```python
from build123d import *

# Parameters (mm, degrees)
EXTRUDE_1_DEPTH     = 680
CUT_EXTRUDE_1_DEPTH = 683.878423476


with BuildPart() as part:
    # 草图1 → 凸台-拉伸1 (new body)
    with BuildSketch(Plane(origin=(0, 0, 0), x_dir=(1, 0, 0), z_dir=(0, 1, 0))):
        with BuildLine():
            Line((-19, -12.278106509), (19, -12.278106509))
            ThreePointArc((19, -12.278106509), (23.242640687, -10.520747196), (25, -6.278106509))
            Line((25, -6.278106509), (25, 31.721893491))
            ThreePointArc((25, 31.721893491), (23.242640687, 35.964534178), (19, 37.721893491))
            Line((19, 37.721893491), (-19, 37.721893491))
            ThreePointArc((-19, 37.721893491), (-23.242640687, 35.964534178), (-25, 31.721893491))
            Line((-25, 31.721893491), (-25, -6.278106509))
            ThreePointArc((-25, -6.278106509), (-23.242640687, -10.520747196), (-19, -12.278106509))
        make_face()
        with BuildLine():
            Line((-19, -7.278106509), (19, -7.278106509))
            ThreePointArc((19, -7.278106509), (19.707106781, -6.98521329), (20, -6.278106509))
            Line((20, -6.278106509), (20, 31.721893491))
            ThreePointArc((20, 31.721893491), (19.707106781, 32.429000272), (19, 32.721893491))
            Line((19, 32.721893491), (-19, 32.721893491))
            ThreePointArc((-19, 32.721893491), (-19.707106781, 32.429000272), (-20, 31.721893491))
            Line((-20, 31.721893491), (-20, -6.278106509))
            ThreePointArc((-20, -6.278106509), (-19.707106781, -6.98521329), (-19, -7.278106509))
        make_face(mode=Mode.SUBTRACT)
    extrude(amount=EXTRUDE_1_DEPTH)

    # 草图2 → 切除-拉伸1 (cut, through all)
    with BuildSketch(Plane(origin=(25, 0, 0), x_dir=(0, 0, -1), z_dir=(1, 0, 0))):
        Polygon((-12.278106509, 680), (37.721893491, 680), (37.721893491, 630), align=None)
        Polygon((-12.278106509, 0), (37.721893491, 50), (37.721893491, 0), align=None)
    extrude(amount=-CUT_EXTRUDE_1_DEPTH, mode=Mode.SUBTRACT)


solid = part.part
```
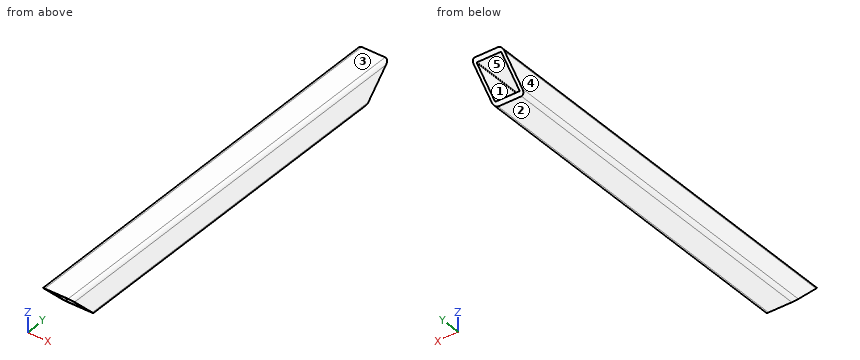
Here's how the part is built. I have some questions about the finished solid (model axes, mm). Face numbers are marked on the shaded views. A direction names the side the tool comes from. Round coordinates to 2 decimals unless told otherwise and drop trailing zeros. Order: outer loops, then holes, each group sorted by start corner. A loop starts at its lowest first (then second) coordinate and runs counter-clockwise, first axis right, second up. Notation, with made-up numbers: M 31,31.25 L 62,31.25 A23 cw 62,42.25 Z; hole C -26,23 d5. An arc over 180 degrees is marked long. Use CSV: the item, a comma, the result in double quotes.
1) I want a section at A-A (x = 0). List the corners of the cut face in (y, z) for me, then the cut area to 3 significant figures.
Taken from the geometry:
outline,"M 0,12.28 L 5,7.28 L 675,7.28 L 680,12.28 Z; M 45,-32.72 L 50,-37.72 L 630,-37.72 L 635,-32.72 Z"
area,"6,300 mm^2"
2) I want a section at B-B (z = -5). List the corners of the cut face in (x, y) for me, then the cut area to 3 significant figures.
Taken from the geometry:
outline,"M -25,17.28 L -20,17.28 L -20,662.72 L -25,662.72 Z; M 20,17.28 L 25,17.28 L 25,662.72 L 20,662.72 Z"
area,"6,450 mm^2"
3) If we mould it in two halves opening along Z, with no side actions, what happens to the marked faces 3, 4 and 5? For each: pulls with the +Z half, pulls with the -Z half, needs draft (parallel to the pull), parting line crosses it, or undercut.
Taken from the geometry:
face 3,"pulls with the +Z half"
face 4,"needs draft"
face 5,"undercut"
4) I need wall thicknesses on line 1 along X through (y, z) = (638, -8.5); line 2 along Z through (x, y) = (-14.5, 176); line 3 along X through (y, z) = (192.5, 9). Which ranges of each line are inside material? Lowest first, please. Write a range as [from, to].
Taken from the geometry:
line 1,"[-25, -20], [20, 25]"
line 2,"[-37.72, -32.72], [7.28, 12.28]"
line 3,"[-24.35, 24.35]"
5) I want a section at C-C (y = 491). List the corners of the cut face in (x, z) for me, then the cut area to 3 significant figures.
Taken from the geometry:
outline,"M -25,-31.72 A6 ccw -19,-37.72 L 19,-37.72 A6 ccw 25,-31.72 L 25,6.28 A6 ccw 19,12.28 L -19,12.28 A6 ccw -25,6.28 Z; hole M -20,-31.72 A1 ccw -19,-32.72 L 19,-32.72 A1 ccw 20,-31.72 L 20,6.28 A1 ccw 19,7.28 L -19,7.28 A1 ccw -20,6.28 Z"
area,"870 mm^2"
6) I'm going to push a flat-ended pin straight in: P1, Ø8, axis at x = -11, z = -29, coming from the +Y side. Where does the tip first touch, or does it pass through?
Taken from the geometry:
P1,"y = 635"
7) On a 3-axis mill with a long thin cutter (end or side, diameter ignored), from which of +Z, -Z, +X, -X, +Y, -Y can I reach the whole of each face in a straight line? I mean the marked faces 1 and 2. Say none if no direction works.
Taken from the geometry:
face 1,"+Y, -Y"
face 2,"-Z, +X, -X, +Y, -Y"
